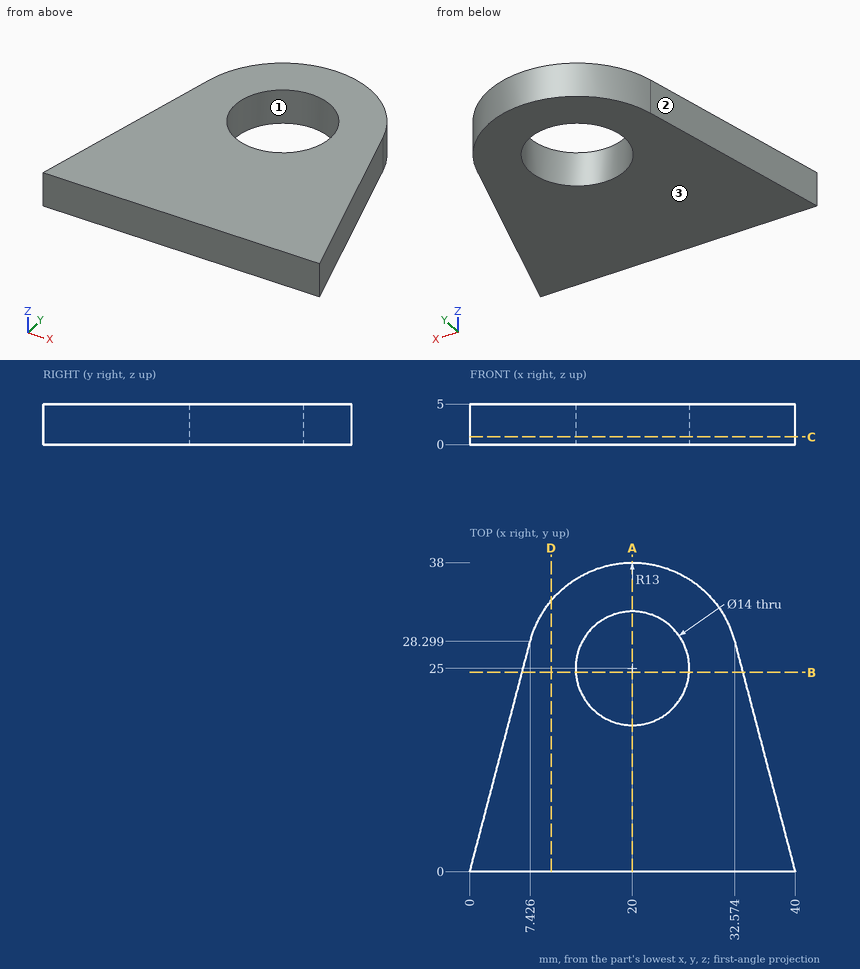
Source: three-view drawing plus pictorial views. Frame: mm from the lowest corner of the part. Round coordinates to 2 decimals unless told otherwise and drop trailing zeros. Loops run counter-clockwise (first coordinate to the right, second up) from the corner with the lowest first, then second, coordinate; pieces in that order, holes last. Notation, with made-up numbers: (41.5, 86) - (92.5, 86) arc R17 ccw to (92.5, 107) - close; hole circle Ø6 at (-11.5, 59.5). An arc over 180 degrees is marked (long way). Write item = value, one per line. Start each with the question number.
Item 1: Section query B-B on y = 24.5. Output: boundary loops of the cut face in (x, z).
Item 2: Material intervals for line 1 (X direction, y = 19, z = 1.5) (1 decimal); line 2 (Y direction, x = 19.5, z = 2.9); line 3 (X direction, y = 22, z = 4.05) (1 decimal), sorted ascending.
Item 3: Section query C-C on z = 0.95. Output: boundary loops of the cut face in (x, y) (1 decimal).
Item 4: Section query A-A on x = 20. Output: boundary loops of the cut face in (y, z).
Item 5: First-contact query: pin 1 Ø8.5 at (x, y) = (20, 25) entering from +Z. Flat tip, straight axial feed; report the tip coordinate or a pass-through.
Item 6: Section query D-D on x = 10. Output: boundary loops of the cut face in (y, z).
Item 7: Mould query, pull axis X, two halves, no side actions, for the marked faces 1, 2 and 3. Classes: released by +X, released by -X, zero draft, split by the parting line, or undercut.
Results list:
q1.outline = (6.43, 0) - (13.02, 0) - (13.02, 5) - (6.43, 5) - close; (26.98, 0) - (33.57, 0) - (33.57, 5) - (26.98, 5) - close
q2.line_1 = 5 to 16.4, 23.6 to 35
q2.line_2 = 0 to 18.02, 31.98 to 37.99
q2.line_3 = 5.8 to 13.7, 26.3 to 34.2
q3.outline = (0, 0) - (40, 0) - (32.6, 28.3) arc R13 ccw to (7.4, 28.3) - close; hole circle Ø14 at (20, 25)
q4.outline = (0, 0) - (18, 0) - (18, 5) - (0, 5) - close; (32, 0) - (38, 0) - (38, 5) - (32, 5) - close
q5.pin_1 = through
q6.outline = (0, 0) - (33.31, 0) - (33.31, 5) - (0, 5) - close
q7.face_1 = undercut
q7.face_2 = released by -X
q7.face_3 = zero draft
